Source: CAD feature listing. Evaluate the final solid. Frame: model axes, mm. A direction names the side the tool comes from. Round coordinates to 2 decimals unless told otherwise and drop trailing zeros. Write each loop counter-clockwise with the first axis right and the second up, starting at its lowest first coordinate (ties: lowest second). Pieces come first, ordered by that corner, then holes.
```python
from build123d import *

# Parameters (mm, degrees)
BOSS_EXTRUDE1_DEPTH          = 10
SKETCH2_W                    = 45
SKETCH2_H                    = 4
F_12_5_12_5_DIAMETER_HOLE1_D = 12.5
M64_CLEARANCE_HOLE1_D        = 70
M64_CLEARANCE_HOLE1_DEPTH    = 4


with BuildPart() as part:
    # Sketch1 → Boss-Extrude1 (new body)
    with BuildSketch(Plane.XY.offset(-144.692981355)):
        with BuildLine():
            Line((511.459420647, 9.123067621), (517.84745191, 53.924775809))
            ThreePointArc((517.84745191, 53.924775809), (387.935069604, 49.592002612), (511.459420647, 9.123067621))
        make_face()
    extrude(amount=-BOSS_EXTRUDE1_DEPTH)

    # Sketch2 → Revolve1 (revolve)
    with BuildSketch(Plane(origin=(0, 40.2756484, 0), x_dir=(1, 0, 0), z_dir=(0, 1, 0))):
        with Locations((475.77422742, 156.692981355)):
            Rectangle(SKETCH2_W, SKETCH2_H)
    revolve(axis=Axis((453.27422742, 40.2756484, -158.692981355), (0, 0, 1)))

    # Ø12.5 (12.5) Diameter Hole1 (through all)
    with Locations(Plane(origin=(0, 0, -154.692981355), x_dir=(-1, 0, 0), z_dir=(0, 0, -1))):
        with Locations((-398.82492924, 48.03927691), (-487.222376026, 83.548309587), (-473.775376995, -10.760641298)):
            Hole(F_12_5_12_5_DIAMETER_HOLE1_D / 2)

    # M64 Clearance Hole1
    with Locations(Plane(origin=(0, 0, -158.692981355), x_dir=(-1, 0, 0), z_dir=(0, 0, -1))):
        with Locations((-453.27422742, 40.2756484)):
            Hole(M64_CLEARANCE_HOLE1_D / 2, depth=M64_CLEARANCE_HOLE1_DEPTH)


solid = part.part
```
Q1. Mould query, pull axis X, two halves, no side actions, for faces 1 (the face through (514.61, 31.21, -149.62)), 2 (the face through (420.11, 70.69, -156.72)), 3 (the face through (467.53, -10.49, -149.62)), 4 (the face through (480, 17, -158.693)). Classes: pulls with the +X half, pulls with the -X half, needs draft (parallel to the pull), parting line crosses it, or undercut.
Q2. Pin query (flat end, axial travel): P1, Ø21, axis at x = 447, y = 51, coming from the -Z side; P2, Ø6, axis at x = 504, z = -152, coming from the +Y side; P3, Ø7.5, axis at x = 398.82, y = 48.04, coming from the -Z side; P4, Ø2, axis at y = -10.5, z = -153, coming from the +X side. Return the tip coordinate at first contact, or that it passes through.
Q3. Set-up query: faces 5 (the face through (490.1, 78, -149.6)), 6 (the face through (418.308, 41.815, -156.665)). Return all of +Z, -Z, +X, -X, +Y, -Y with unobstructed straight access to the full face (end or side cutting, diameter ignored); none if empty.
Q4. Section query B-B, the plane x = 483. Output: boundary loops of the cut face in (y, z).
Q5. Line query: line 1 (Z direction, x = 439, y = 33.5); line 2 (X direction, y = -8, z = -145.75); line 3 (Y direction, x = 447.5, z = -154.75). Output: solid intervals per line, ascending.
Q6. Section query D-D, the plane y = 26. Output: boundary loops of the cut face in (x, z).
Q7. Section query C-C, the plane z = -152.5. Output: boundary loops of the cut face in (x, y).
Q8. Section query A-A, the plane y = 46. Output: boundary loops of the cut face in (x, z), and give its area (3 significant figures).
Filled in:
1. face 1: pulls with the +X half
1. face 2: parting line crosses it
1. face 3: undercut
1. face 4: needs draft
2. P1: stops at z = -154.69
2. P2: stops at y = 85.86
2. P3: passes through
2. P4: stops at x = 496.61
3. face 5: +Z, -Z
3. face 6: -Z
4. outline: (-18.65, -154.69) - (6.49, -154.69) - (6.49, -158.69) - (21.8, -158.69) - (21.8, -154.69) - (58.75, -154.69) - (58.75, -158.69) - (74.06, -158.69) - (74.06, -154.69) - (78.94, -154.69) - (78.94, -144.69) - (-18.65, -144.69) - close; (88.16, -154.69) - (99.2, -154.69) - (99.2, -144.69) - (88.16, -144.69) - close
5. line 1: z = -154.69 to -144.69
5. line 2: x = 408.27 to 468.17, 479.38 to 498.28
5. line 3: y = -4.35 to 5.76, 74.8 to 84.9
6. outline: (388.84, -154.69) - (410.6, -154.69) - (410.6, -158.69) - (421.32, -158.69) - (421.32, -154.69) - (485.23, -154.69) - (485.23, -158.69) - (495.95, -158.69) - (495.95, -154.69) - (513.87, -154.69) - (513.87, -144.69) - (388.84, -144.69) - close
7. outline: (511.46, 9.12) - (517.85, 53.92) arc R66 ccw (long way) to start; hole circle Ø12.5 at (398.82, 48.04); hole circle Ø12.5 at (473.78, -10.76); hole circle Ø12.5 at (487.22, 83.55)
8. outline: (387.52, -154.69) - (392.92, -154.69) - (392.92, -144.69) - (387.52, -144.69) - close; (404.73, -154.69) - (408.64, -154.69) - (408.64, -158.69) - (418.75, -158.69) - (418.75, -154.69) - (487.8, -154.69) - (487.8, -158.69) - (497.91, -158.69) - (497.91, -154.69) - (516.72, -154.69) - (516.72, -144.69) - (404.73, -144.69) - close
8. area: 1,250 mm2
